Design review of the part built by this model. Coordinates are the model's own, in mm. Face numbers are marked on the shaded views. A direction names the side the tool comes from. Give positions to 0.01 mm unless a question says otherwise; leave off trailing zeros. Order: outer loops, then holes, each group sorted by start corner. A loop starts at its lowest first (then second) coordinate and runs counter-clockwise, first axis right, second up. Notation, with made-up numbers: (67.5, 78.25) -> (86.5, 78.25) arc R14 cw to (86.5, 95.25) -> close; hole circle Ø7 at (-17.75, 26). An arc over 180 degrees is marked (long way). Return JSON: item names as keys, results as strings.
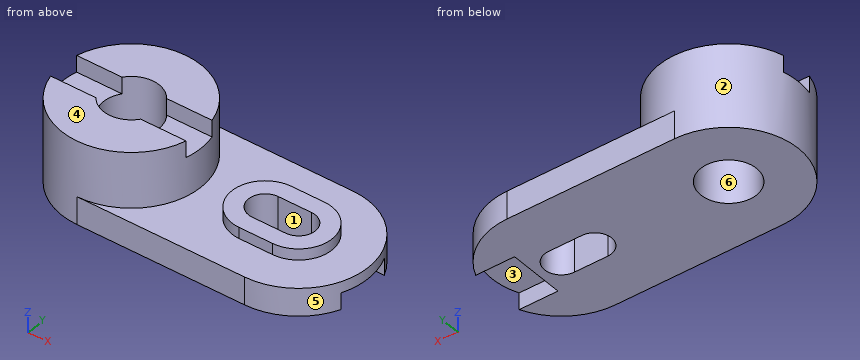
```python
from build123d import *

# Parameters (mm, degrees)
ARM_PLATE_DEPTH      = 10
HUB_FRONT_SKETCH_R   = 25
HUB_BOSS_FRONT_DEPTH = 10
HUB_START            = 20
HUB_BACK_SKETCH_R    = 25
HUB_BOSS_BACK_DEPTH  = 20
HUB_CROSS_SLOT_DEPTH = 6
BORE_SKETCH_R        = 10
BORE_20_DEPTH        = 30
SLOT_BOSS_DEPTH      = 4
ARM_SLOT_12MM_DEPTH  = 20
END_NOTCH_DEPTH      = 94.541434669
END_NOTCH_DEPTH_BACK = 6


with BuildPart() as part:
    # Arm Profile Sketch → Arm Plate (new body)
    with BuildSketch(Plane.XY):
        with BuildLine():
            Line((60, 25), (0, 25))
            Line((0, 25), (0, -25))
            Line((0, -25), (60, -25))
            ThreePointArc((60, -25), (85, 0), (60, 25))
        make_face()
    extrude(amount=ARM_PLATE_DEPTH)

    # Hub Front Sketch → Hub Boss Front (add)
    with BuildSketch(Plane.XY.offset(10)):
        Circle(HUB_FRONT_SKETCH_R)
    extrude(amount=-HUB_BOSS_FRONT_DEPTH)

    # Hub Back Sketch → Hub Boss Back (add)
    with BuildSketch(Plane.XY.offset(10).offset(HUB_START)):
        Circle(HUB_BACK_SKETCH_R)
    extrude(amount=-HUB_BOSS_BACK_DEPTH)

    # Hub Cross Slot Sketch → Hub Cross Slot (cut)
    with BuildSketch(Plane.XY.offset(30)):
        with BuildLine():
            ThreePointArc((24.269322199, -6), (24.816658266, -3.022163548), (25, 0))
            ThreePointArc((25, 0), (24.816658266, 3.022163548), (24.269322199, 6))
            Line((24.269322199, 6), (8, 6))
            ThreePointArc((8, 6), (0, 10), (-8, 6))
            Line((-8, 6), (-24.269322199, 6))
            ThreePointArc((-24.269322199, 6), (-24.816658266, 3.022163548), (-25, 0))
            ThreePointArc((-25, 0), (-24.816658266, -3.022163548), (-24.269322199, -6))
            Line((-24.269322199, -6), (-8, -6))
            ThreePointArc((-8, -6), (0, -10), (8, -6))
            Line((8, -6), (24.269322199, -6))
        make_face()
    extrude(amount=-HUB_CROSS_SLOT_DEPTH, mode=Mode.SUBTRACT)

    # Bore Sketch → Bore Ø20 (cut)
    with BuildSketch(Plane.XY.offset(24)):
        Circle(BORE_SKETCH_R)
    extrude(amount=-BORE_20_DEPTH, mode=Mode.SUBTRACT)

    # Slot Boss Sketch → Slot Boss (add)
    with BuildSketch(Plane.XY.offset(10)):
        with BuildLine():
            Line((48, 12), (60, 12))
            ThreePointArc((60, 12), (72, 0), (60, -12))
            Line((60, -12), (48, -12))
            ThreePointArc((48, -12), (36, 0), (48, 12))
        make_face()
    extrude(amount=SLOT_BOSS_DEPTH)

    # Arm Slot Sketch → Arm Slot 12mm (cut)
    with BuildSketch(Plane.XY.offset(14)):
        with BuildLine():
            Line((48, 6), (60, 6))
            ThreePointArc((60, 6), (66, 0), (60, -6))
            Line((60, -6), (48, -6))
            ThreePointArc((48, -6), (42, 0), (48, 6))
        make_face()
    extrude(amount=-ARM_SLOT_12MM_DEPTH, mode=Mode.SUBTRACT)

    # End Notch Sketch → End Notch (cut, two sides: drawn at the far end of the back side and taken through both)
    with BuildSketch(Plane(origin=(0, 0, 0), x_dir=(-1, 0, 0), z_dir=(0, 0, -1)).offset(-END_NOTCH_DEPTH_BACK)):
        Polygon((-319.806592277, -10), (-82.912878475, -10), (-79, -10), (-69, -10), (-69, 10), (-79, 10), (-82.912878475, 10), (-319.806592277, 10), (-793.594019881, 10), (-793.594019881, -10), align=None)
    extrude(amount=END_NOTCH_DEPTH + END_NOTCH_DEPTH_BACK, mode=Mode.SUBTRACT)


solid = part.part
```
Item 1: Add section D-D (y = 13). Give the boundary of the cut face in (x, z).
Result set:
{"outline": "(-21.35, 0) -> (81.35, 0) -> (81.35, 10) -> (21.35, 10) -> (21.35, 30) -> (-21.35, 30) -> close"}
Item 2: Wall thickness on L1, parallel to X at y = 0, z = 12; L2, parallel to Y at x = 0, z = 13.75: over which ranges is each line inside the solid? List them lowest first. Write a range as [from, to].
Result set:
{"L1": "x = [-25, -10], [10, 25], [36, 42], [66, 72]", "L2": "y = [-25, -10], [10, 25]"}
Item 3: Add section C-C (z = 21). Give the boundary of the cut face in (x, y), plus the area to 3 significant figures.
Result set:
{"outline": "circle Ø50 at (0, 0); hole circle Ø20 at (0, 0)", "area": "1,650 mm^2"}
Item 4: Add section B-B (x = 12). Give the boundary of the cut face in (y, z), plus the area to 3 significant figures.
Result set:
{"outline": "(-25, 0) -> (25, 0) -> (25, 10) -> (21.93, 10) -> (21.93, 30) -> (6, 30) -> (6, 24) -> (-6, 24) -> (-6, 30) -> (-21.93, 30) -> (-21.93, 10) -> (-25, 10) -> close", "area": "1,310 mm^2"}
Item 5: Mouldability with a two-part tool opening along X and no side actions: class the marked faces 4, 5 and 6 as released by +X, released by -X, zero draft, split by the parting line, or undercut.
Result set:
{"face 4": "zero draft", "face 5": "released by +X", "face 6": "undercut"}
Item 6: For pin 1 (1.8 mm diameter, centred on x = -18, z = 26.5, fed in from +Y); pin 2 (4.5 mm diameter, centred on x = 55, z = 12.5, fed in from -Y); pin 3 (12 mm diameter, centred on y = 19.5, z = 26.5, fed in from +X), all flat-tipped, find the tip position at first contact; note any pin that passes through.
Result set:
{"pin 1": "stops at y = 18.24", "pin 2": "stops at y = -12", "pin 3": "stops at x = 21.04"}
Item 7: Add section A-A (y = 0). Give the boundary of the cut face in (x, z), plus the area to 3 significant figures.
Result set:
{"outline": "(-25, 0) -> (-10, 0) -> (-10, 24) -> (-25, 24) -> close; (10, 0) -> (42, 0) -> (42, 14) -> (36, 14) -> (36, 10) -> (25, 10) -> (25, 24) -> (10, 24) -> close; (66, 0) -> (69, 0) -> (69, 6) -> (85, 6) -> (85, 10) -> (72, 10) -> (72, 14) -> (66, 14) -> close", "area": "1,030 mm^2"}
Item 8: Machinability: for the marked faces 1, 2 and 3, which of the approach directions +Z, -Z, +X, -X, +Y, -Y give a long, thin tool a straight path to every point of the face, cutting with its end or side? Answer none if there is none.
Result set:
{"face 1": "+Z, -Z", "face 2": "+Z", "face 3": "-Z, +X"}
